Part model, mm, in its own coordinate system. Face numbers are marked on the shaded views. A direction names the side the tool comes from. Round coordinates to 2 decimals unless told otherwise and drop trailing zeros. Order: outer loops, then holes, each group sorted by start corner. A loop starts at its lowest first (then second) coordinate and runs counter-clockwise, first axis right, second up. Notation, with made-up numbers: (1.5, 28) - (46.5, 28) arc R35 ccw to (46.5, 62) - close; hole circle Ø11 at (36, 89.25). An arc over 180 degrees is marked (long way). Answer as a JSON object with one key per item and string values.
```python
from build123d import *

# Parameters (mm, degrees)
BOSS_EXTRUDE1_DEPTH = 18


with BuildPart() as part:
    # Sketch1 → Boss-Extrude1 (new body)
    with BuildSketch(Plane.XY):
        with BuildLine():
            Line((0, 0), (0, 100))
            Line((0, 100), (55, 100))
            Line((55, 100), (55, 95.82575695))
            ThreePointArc((55, 95.82575695), (33.166998673, 77.386127875), (25, 50))
            Line((25, 50), (25, 0))
            Line((25, 0), (0, 0))
        make_face()
    extrude(amount=BOSS_EXTRUDE1_DEPTH)


solid = part.part
```
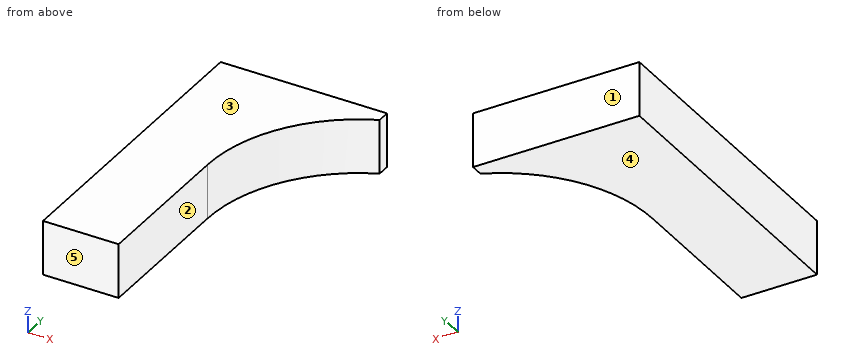
Item 1: Cut at C-C (x = 46.5). Write the cut outline in (y, z), plus the area to 3 significant figures.
Taken from the geometry:
{"outline": "(91.08, 0) - (100, 0) - (100, 18) - (91.08, 18) - close", "area": "161 mm2"}
Item 2: Two-plate mould, pull along Z, no slides. Class the marked faces 3, 4 and 5: pulls with the +Z half, pulls with the -Z half, needs draft (parallel to the pull), parting line crosses it, or undercut.
Taken from the geometry:
{"face 3": "pulls with the +Z half", "face 4": "pulls with the -Z half", "face 5": "needs draft"}
Item 3: Cut at B-B (y = 80). Write the cut outline in (x, z).
Taken from the geometry:
{"outline": "(0, 0) - (35, 0) - (35, 18) - (0, 18) - close"}
Item 4: Drop flat-ended pins along their axis: P1, Ø6, axis at x = 44.5, z = 4, coming from the -Y side; P2, Ø6, axis at x = 47, z = 4, coming from the -Y side; P3, Ø4, axis at x = 46.5, z = 4.5, coming from the -Y side. Give the stop position or say it passes through.
Taken from the geometry:
{"P1": "y = 87.12", "P2": "y = 89.23", "P3": "y = 89.62"}
Item 5: Probe L1, parallel to X at y = 51, z = 8; L2, parallel to X at y = 87, z = 11; L3, parallel to Y at x = 39.5, z = 13. List the from-to ranges inside material, lowest first. Write a range as from..to.
Taken from the geometry:
{"L1": "0..25.01", "L2": "0..41.37", "L3": "85.21..100"}
Item 6: Tool access for the marked faces 1 and 2: list every direction of +Z, -Z, +X, -X, +Y, -Y with a clear straight run to the whole face (end or side of a thin tool).
Taken from the geometry:
{"face 1": "+Z, -Z, +X, -X, +Y", "face 2": "+Z, -Z, +X, -Y"}
Item 7: Cut at A-A (z = 5). Write the cut outline in (x, y), plus the area to 3 significant figures.
Taken from the geometry:
{"outline": "(0, 0) - (25, 0) - (25, 50) arc R50 cw to (55, 95.83) - (55, 100) - (0, 100) - close", "area": "3,010 mm2"}
